```python
from build123d import *

# Parameters (mm, degrees)
BASE_BLOCK_DEPTH              = 31
STEPPED_CHANNEL_THROUGH_DEPTH = 62
TOP_SLOT_POCKET_12_DEEP_DEPTH = 12
BOTTOM_GROOVE_SKETCH_W        = 50
BOTTOM_GROOVE_SKETCH_H        = 6
BOTTOM_GROOVE_6X6_DEPTH       = 114.564959384


with BuildPart() as part:
    # Base Profile Sketch → Base Block (new, symmetric)
    with BuildSketch(Plane.XY):
        Polygon((0, 0), (0, 26), (63, 26), (63, 44), (100, 44), (100, 0), align=None)
    extrude(amount=BASE_BLOCK_DEPTH, both=True)

    # Stepped Channel Sketch → Stepped Channel Through (cut)
    with BuildSketch(Plane(origin=(0, 26, 0), x_dir=(1, 0, 0), z_dir=(0, 1, 0))):
        with BuildLine():
            Line((23, 8), (43, 8))
            ThreePointArc((43, 8), (51, 0), (43, -8))
            Line((43, -8), (23, -8))
            ThreePointArc((23, -8), (15, 0), (23, 8))
        make_face()
    extrude(amount=-STEPPED_CHANNEL_THROUGH_DEPTH, mode=Mode.SUBTRACT)

    # Top Slot Sketch → Top Slot Pocket 12 Deep (cut)
    with BuildSketch(Plane(origin=(0, 44, 0), x_dir=(1, 0, 0), z_dir=(0, 1, 0))):
        Polygon((63, 18.5), (63, -18.5), (100, -12.5), (100, 12.5), align=None)
    extrude(amount=-TOP_SLOT_POCKET_12_DEEP_DEPTH, mode=Mode.SUBTRACT)

    # Bottom Groove Sketch → Bottom Groove 6x6 (cut, through all)
    with BuildSketch(Plane.ZY):
        with Locations((0, 3)):
            Rectangle(BOTTOM_GROOVE_SKETCH_W, BOTTOM_GROOVE_SKETCH_H)
    extrude(amount=-BOTTOM_GROOVE_6X6_DEPTH, mode=Mode.SUBTRACT)


solid = part.part
```
Here's how the part is built. I have some questions about the finished solid (model axes, mm). A direction names the side the tool comes from. Round coordinates to 2 decimals unless told otherwise and drop trailing zeros. Loops run counter-clockwise (first coordinate to the right, second up) from the corner with the lowest first, then second, coordinate; pieces in that order, holes last. Notation, with made-up numbers: (-13.5, 71.25) -> (13.5, 71.25) arc R18 ccw to (13.5, 79.25) -> close; hole circle Ø8 at (65.5, 15.5). An arc over 180 degrees is marked (long way). Answer as CSV lines item,"result". Start each with the question number.
1. If we mould it in two halves opening along Z, with no side actions, what happens to faces 4 (the face through (31, 26, 14)), 5 (the face through (81.759, 38.084, -15.458)), 6 (the face through (62, 17, 31)), 7 (the face through (62, 17, -31))? For each: pulls with the +Z half, pulls with the -Z half, needs draft (parallel to the pull), parting line crosses it, or undercut.
2. Imagine slicing it at A-A on y = 40. Write out the boundary of the cut face in (x, z).
3. For faces 1 (the face through (49, 3, 25)), 2 (the face through (33, 16, 8)), 3 (the face through (63, 31, 0)), which set-ups out of +Z, -Z, +X, -X, +Y, -Y let a thin tool reach every point of the face, with its end or its side?
4. Imagine slicing it at B-B on z = 0. Write out the boundary of the cut face in (x, y).
5. Imagine slicing it at D-D on x = 53. Write out the boundary of the cut face in (y, z).
6. Imagine slicing it at C-C on y = 14. Write out the boundary of the cut face in (x, z).
7. I'm going to push flat-ended pins straight in: P1, Ø18.5, axis at x = 35.5, z = 3, coming from the +Y side; P2, Ø10, axis at x = 19, z = 12.5, coming from the -Y side; P3, Ø10, axis at x = 75, z = -15.5, coming from the +Y side. Where does each tip first touch, or does it pass through?
8. I need wall thicknesses on probe 1 along Y at (x, z) = (44.5, -22.5); probe 2 along Z at (x, y) = (23.5, 23); probe 3 along Y at (x, z) = (50.5, 27). Which ranges of each line are inside material? Lowest first, please. Write a range as from..to.
Solution:
1,face 4,"needs draft"
1,face 5,"undercut"
1,face 6,"pulls with the +Z half"
1,face 7,"pulls with the -Z half"
2,outline,"(63, -31) -> (100, -31) -> (100, -12.5) -> (63, -18.5) -> close; (63, 18.5) -> (100, 12.5) -> (100, 31) -> (63, 31) -> close"
3,face 1,"+X, -X, -Y"
3,face 2,"+Y, -Y"
3,face 3,"+Z, -Z, -X, +Y"
4,outline,"(0, 6) -> (15, 6) -> (15, 26) -> (0, 26) -> close; (51, 6) -> (100, 6) -> (100, 32) -> (63, 32) -> (63, 26) -> (51, 26) -> close"
5,outline,"(0, -31) -> (26, -31) -> (26, 31) -> (0, 31) -> (0, 25) -> (6, 25) -> (6, -25) -> (0, -25) -> close"
6,outline,"(0, -31) -> (100, -31) -> (100, 31) -> (0, 31) -> close; hole (23, -8) -> (43, -8) arc R8 ccw to (43, 8) -> (23, 8) arc R8 ccw to start"
7,P1,"y = 26"
7,P2,"y = 6"
7,P3,"y = 44"
8,probe 1,"6..26"
8,probe 2,"-31..-8, 8..31"
8,probe 3,"0..26"
